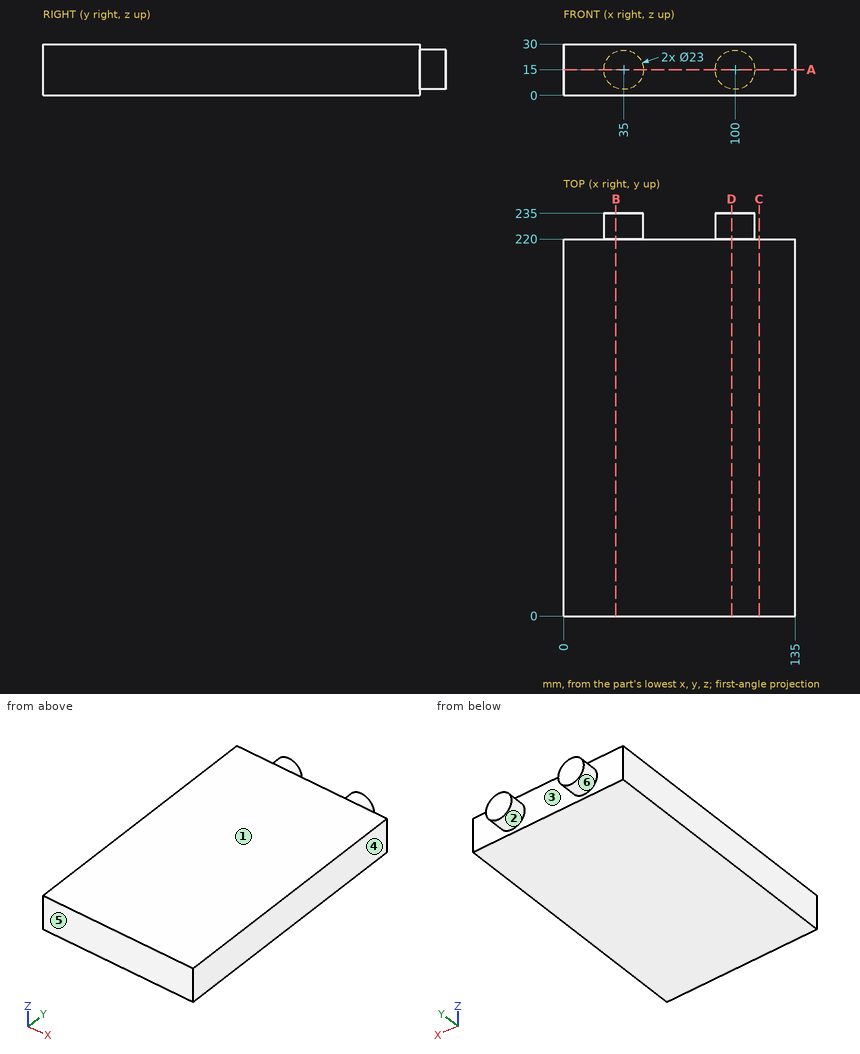
The drawing under review shows one solid part. Ordinate dimensions are in mm from its lowest x, y, z. A direction names the side the tool comes from. Coordinates: 2 decimals unless noted, no trailing zeros. Loops run counter-clockwise (first coordinate to the right, second up) from the corner with the lowest first, then second, coordinate; pieces in that order, holes last. Notation, with made-up numbers: (70.25, 78) - (99.25, 78) arc R23 ccw to (99.25, 115) - close; hole circle Ø8 at (-12.75, 20). An arc over 180 degrees is marked (long way). Return JSON: item names as keys, results as strings.
Item 1: Mouldability with a two-part tool opening along X and no side actions: class the marked faces 3, 4, 5 and 6 as pulls with the +X half, pulls with the -X half, needs draft (parallel to the pull), parting line crosses it, or undercut.
Determined:
{"face 3": "undercut", "face 4": "pulls with the +X half", "face 5": "needs draft", "face 6": "undercut"}
Item 2: Take a section at D-D (x = 98). Give the boundary of the cut face in (y, z).
Determined:
{"outline": "(0, 0) - (220, 0) - (220, 3.68) - (235, 3.68) - (235, 26.32) - (220, 26.32) - (220, 30) - (0, 30) - close"}
Item 3: For line 1 (Y direction, x = 105, z = 26), list the stretches that pass through material, from the lowest coordinate up.
Determined:
{"line 1": "y = 0 to 220"}
Item 4: Take a section at B-B (x = 30.5). Give the boundary of the cut face in (y, z), then the cut area to 3 significant figures.
Determined:
{"outline": "(0, 0) - (220, 0) - (220, 4.42) - (235, 4.42) - (235, 25.58) - (220, 25.58) - (220, 30) - (0, 30) - close", "area": "6,920 mm2"}
Item 5: Take a section at C-C (x = 114). Give the boundary of the cut face in (y, z), then the cut area to 3 significant figures.
Determined:
{"outline": "(0, 0) - (220, 0) - (220, 30) - (0, 30) - close", "area": "6,600 mm2"}
Item 6: Take a section at A-A (z = 15). Give the boundary of the cut face in (x, y), then the cut area to 3 significant figures.
Determined:
{"outline": "(0, 0) - (135, 0) - (135, 220) - (111.5, 220) - (111.5, 235) - (88.5, 235) - (88.5, 220) - (46.5, 220) - (46.5, 235) - (23.5, 235) - (23.5, 220) - (0, 220) - close", "area": "30,400 mm2"}
Item 7: For the marked faces 1 and 2, list the 3-axis set-ups (+Z, -Z, +X, -X, +Y, -Y) from which the entire face can be reached by the end or side of a thin tool; tool diameter is ignored.
Determined:
{"face 1": "+Z, +X, -X, +Y, -Y", "face 2": "+Y"}
Item 8: Insertion check: pin 1 (12 mm diameter, centred on x = 118, z = 16, fed in from +Y). The pin has a flat end and moves straight along its axis. Give the tip position at first contact, or say it passes through.
Determined:
{"pin 1": "stops at y = 220"}
